Answer from the drawing. Dimensions are ordinates in mm from the lowest x, y and z of the part. Round coordinates to 2 decimals unless told otherwise and drop trailing zeros. Loops run counter-clockwise (first coordinate to the right, second up) from the corner with the lowest first, then second, coordinate; pieces in that order, holes last.
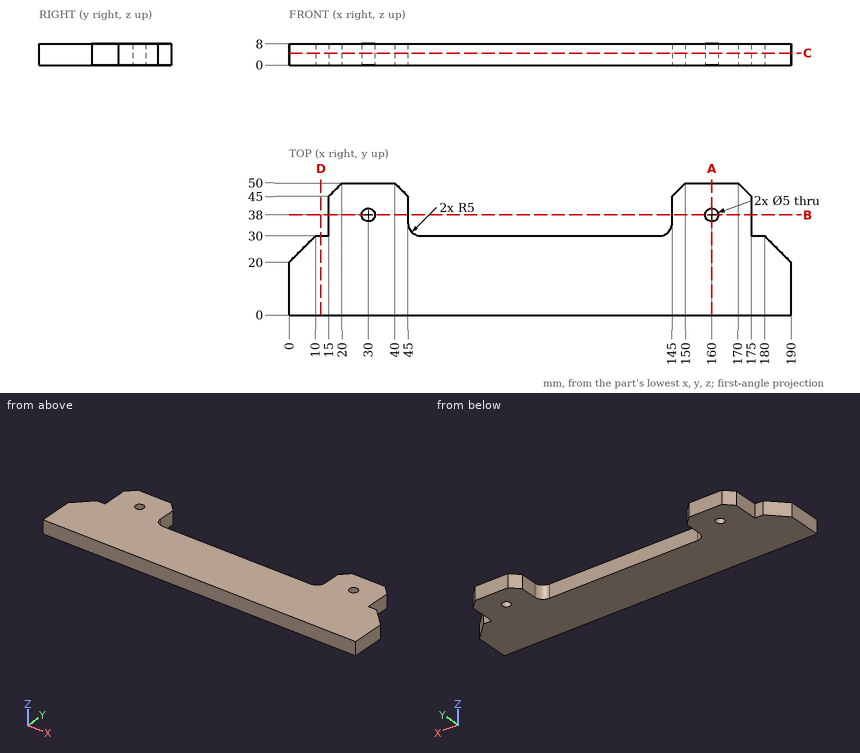
1. Find section C-C (z = 4.5). Write down the section's boundary in (x, y), then the cut area to 3 significant figures.
Answer key:
outline: (0, 0) - (190, 0) - (190, 20) - (180, 30) - (175, 30) - (175, 45) - (170, 50) - (150, 50) - (145, 45) - (145, 35) arc R5 cw to (140, 30) - (50, 30) arc R5 cw to (45, 35) - (45, 45) - (40, 50) - (20, 50) - (15, 45) - (15, 30) - (10, 30) - (0, 20) - close; hole circle Ø5 at (30, 38); hole circle Ø5 at (160, 38)
area: 6,720 mm2
2. Find section B-B (y = 38). Write down the section's boundary in (x, z), then the cut area to 3 significant figures.
Answer key:
outline: (15, 0) - (27.5, 0) - (27.5, 8) - (15, 8) - close; (32.5, 0) - (45, 0) - (45, 8) - (32.5, 8) - close; (145, 0) - (157.5, 0) - (157.5, 8) - (145, 8) - close; (162.5, 0) - (175, 0) - (175, 8) - (162.5, 8) - close
area: 400 mm2
3. Consider probe 1 along X at (y, z) = (34.5, 3); probe 2 along Y at (x, z) = (30, 5.5); probe 3 along Y at (x, z) = (112, 7.25). Determine where each line is inside the solid, lowest interval first.
Answer key:
probe 1: x = 15 to 45.03, 144.97 to 175
probe 2: y = 0 to 35.5, 40.5 to 50
probe 3: y = 0 to 30
4. Find section A-A (x = 160). Write down the section's boundary in (y, z), then the cut area to 3 significant figures.
Answer key:
outline: (0, 0) - (35.5, 0) - (35.5, 8) - (0, 8) - close; (40.5, 0) - (50, 0) - (50, 8) - (40.5, 8) - close
area: 360 mm2
5. Given pin 1 (4 mm diameter, centred on y = 31, z = 2.5, fed in from +X); pin 2 (2.5 mm diameter, centred on x = 12.5, z = 4.5, fed in from +Y); pin 3 (2.5 mm diameter, centred on y = 39.5, z = 2, fed in from +X); pin 4 (4 mm diameter, centred on x = 30, y = 38, fed in from -Z), each flat-ended and moving along its own axis, determine where each tip first touches the part or whether it passes through.
Answer key:
pin 1: stops at x = 181
pin 2: stops at y = 30
pin 3: stops at x = 175
pin 4: passes through
6. Find section D-D (x = 12). Write down the section's boundary in (y, z), then the cut area to 3 significant figures.
Answer key:
outline: (0, 0) - (30, 0) - (30, 8) - (0, 8) - close
area: 240 mm2
